The model under review builds one solid part; all positions refer to its coordinate system, in mm. A direction names the side the tool comes from. Round coordinates to 2 decimals unless told otherwise and drop trailing zeros. Loops run counter-clockwise (first coordinate to the right, second up) from the corner with the lowest first, then second, coordinate; pieces in that order, holes last. Notation, with made-up numbers: M -12,84 L 22,84 A15 cw 22,109 Z; hole C 25.5,14.5 d3. An arc over 180 degrees is marked long. Answer in a Markdown table with one row per item. Add a question column.
from build123d import *

# Parameters (mm, degrees)
BASE_PROFILE_SKETCH_R                = 7
BASE_BLOCK_DEPTH                     = 55
GUIDE_SLOT_SKETCH_W                  = 28
GUIDE_SLOT_SKETCH_H                  = 78
GUIDE_SLOT_16X16_DEPTH               = 110
PIVOT_LUG_SKETCH_R                   = 10
PIVOT_LUG_DEPTH                      = 12
LUG_SUPPORT_SKETCH_R                 = 22.5
LUG_SUPPORT_SKETCH_R_2               = 10
LUG_SUPPORT_BOSS_DEPTH               = 8
COUNTERBORED_HOLES_3X_12_D           = 12
COUNTERBORED_HOLES_3X_12_DEPTH       = 99.819837708
COUNTERBORED_HOLES_3X_12_CBORE_D     = 24
COUNTERBORED_HOLES_3X_12_CBORE_DEPTH = 6


with BuildPart() as part:
    # Base Profile Sketch → Base Block (new, symmetric)
    with BuildSketch(Plane.XY):
        with BuildLine():
            Line((0, -14), (56, -14))
            Line((56, -14), (56, 3.5))
            Line((56, 3.5), (76, 3.5))
            Line((76, 3.5), (76, -14))
            Line((76, -14), (96, -14))
            Line((96, -14), (96, 21))
            Line((96, 21), (36, 21))
            Line((36, 21), (36, 36))
            Line((36, 36), (24, 36))
            Line((24, 36), (-8.50921229, 11.117252638))
            ThreePointArc((-8.50921229, 11.117252638), (-13.259742398, -4.492129955), (0, -14))
        make_face()
        Circle(BASE_PROFILE_SKETCH_R, mode=Mode.SUBTRACT)
    extrude(amount=BASE_BLOCK_DEPTH, both=True)

    # Guide Slot Sketch → Guide Slot 16x16 (cut)
    with BuildSketch(Plane.XZ.offset(14)):
        Rectangle(GUIDE_SLOT_SKETCH_W, GUIDE_SLOT_SKETCH_H)
    extrude(amount=-GUIDE_SLOT_16X16_DEPTH, mode=Mode.SUBTRACT)

    # Pivot Lug Sketch → Pivot Lug (add)
    with BuildSketch(Plane(origin=(36, 0, 0), x_dir=(0, 0, -1), z_dir=(1, 0, 0))):
        with BuildLine():
            Line((35, 36), (21.299956881, 76.249954267))
            ThreePointArc((21.299956881, 76.249954267), (0, 91.5), (-21.299956881, 76.249954267))
            Line((-21.299956881, 76.249954267), (-35, 36))
            Line((-35, 36), (35, 36))
        make_face()
        with Locations((0, 69)):
            Circle(PIVOT_LUG_SKETCH_R, mode=Mode.SUBTRACT)
    extrude(amount=-PIVOT_LUG_DEPTH)

    # Lug Support Sketch → Lug Support Boss (add)
    with BuildSketch(Plane.ZY.offset(-24)):
        with Locations(Location((0, 69, 0), (0, 0, 161.202754194))):
            Circle(LUG_SUPPORT_SKETCH_R)
        with Locations(Location((0, 69, 0), (0, 0, 180))):
            Circle(LUG_SUPPORT_SKETCH_R_2, mode=Mode.SUBTRACT)
    extrude(amount=LUG_SUPPORT_BOSS_DEPTH)

    # Counterbored Holes 3xØ12
    with Locations(Plane(origin=(66, 21, 35), x_dir=(1, 0, 0), z_dir=(0, 1, 0))):
        with Locations((0, 0), (0, 35), (0, 70)):
            CounterBoreHole(COUNTERBORED_HOLES_3X_12_D / 2, COUNTERBORED_HOLES_3X_12_CBORE_D / 2, COUNTERBORED_HOLES_3X_12_CBORE_DEPTH, depth=COUNTERBORED_HOLES_3X_12_DEPTH)


solid = part.part
1. Take a section at B-B, the plane y = 0. State the section outline as (x, z) points, and give its area (3 significant figures).
2. For pin 1 Ø9 at (y, z) = (-5, -9) entering from -X; pin 2 Ø4 at (y, z) = (78.5, 3.5) entering from +X; pin 3 Ø13 at (x, z) = (27.5, -44.5) entering from +Y, all flat-tipped, find the tip position at first contact; note any pin that passes through.
3. Take a section at A-A, the plane z = 0. State the section outline as (x, y) points.
4. Take a section at C-C, the plane x = 66. State the section outline as (y, z) points, and give its area (3 significant figures).
5. Mouldability with a two-part tool opening along Z and no side actions: class faces 5 (the flat face through (40, 6, 55)), 6 (the flat face through (96, 3, 1)), 7 (the flat face through (60, 15, 37)) as released by +Z, released by -Z, zero draft, split by the parting line, or undercut.
6. Take a section at D-D, the plane y = 69. State the section outline as (x, z) points.
7. Machinability: for faces 1 (the cylindrical face through (57.156, 18.042, 26.89)), 2 (the flat face through (30, 36, -45)), 3 (the flat face through (30, 36, 45)), 4 (the flat face through (14, 7, -1)), which of the approach directions +Z, -Z, +X, -X, +Y, -Y give a long, thin tool a straight path to every point of the face, cutting with its end or side? Answer none if there is none.
8. To check wall thickness, follow probe 1 along Z at (x, y) = (66, 11); probe 2 along X at (y, z) = (-0.5, -49.5); probe 3 along X at (y, z) = (18, -35). State the ranges of each line that lie inside material, in increasing order.
Check sheet entries:
| question | item | result |
|---|---|---|
| 1 | outline | M -14,-55 L -7,-55 L -7,-39 L -14,-39 Z; M -14,39 L -7,39 L -7,55 L -14,55 Z; M 7,-55 L 56,-55 L 56,55 L 7,55 L 7,39 L 14,39 L 14,-39 L 7,-39 Z; M 76,-55 L 96,-55 L 96,55 L 76,55 Z |
| 1 | area | 7,270 mm^2 |
| 2 | pin 1 | stops at x = 14 |
| 2 | pin 2 | stops at x = 36 |
| 2 | pin 3 | stops at y = 36 |
| 3 | outline | M 14,-14 L 56,-14 L 56,3.5 L 60,3.5 L 60,15 L 54,15 L 54,21 L 36,21 L 36,59 L 16,59 L 16,46.5 L 24,46.5 L 24,36 L 14,28.35 Z; M 16,79 L 36,79 L 36,91.5 L 16,91.5 Z; M 72,3.5 L 76,3.5 L 76,-14 L 96,-14 L 96,21 L 78,21 L 78,15 L 72,15 Z |
| 4 | outline | M 3.5,-55 L 21,-55 L 21,-47 L 15,-47 L 15,-41 L 3.5,-41 Z; M 3.5,-29 L 15,-29 L 15,-23 L 21,-23 L 21,-12 L 15,-12 L 15,-6 L 3.5,-6 Z; M 3.5,6 L 15,6 L 15,12 L 21,12 L 21,23 L 15,23 L 15,29 L 3.5,29 Z; M 3.5,41 L 15,41 L 15,47 L 21,47 L 21,55 L 3.5,55 Z |
| 4 | area | 1,080 mm^2 |
| 5 | face 5 | released by +Z |
| 5 | face 6 | zero draft |
| 5 | face 7 | undercut |
| 6 | outline | M 16,-22.5 L 24,-22.5 L 24,-23.77 L 36,-23.77 L 36,-10 L 16,-10 Z; M 16,10 L 36,10 L 36,23.77 L 24,23.77 L 24,22.5 L 16,22.5 Z |
| 7 | face 1 | +Y |
| 7 | face 2 | -Z, +X, -X, +Y |
| 7 | face 3 | +Z, +X, -X, +Y |
| 7 | face 4 | -X, +Y, -Y |
| 8 | probe 1 | z = -55 to -41, -29 to -6, 6 to 29, 41 to 55 |
| 8 | probe 2 | x = -13.99 to -6.98, 6.98 to 56, 76 to 96 |
| 8 | probe 3 | x = 14 to 54, 78 to 96 |
